For this review, take the finished solid that the model builds, in its own axes (mm). A direction names the side the tool comes from. Coordinates: 2 decimals unless noted, no trailing zeros. Order: outer loops, then holes, each group sorted by start corner. A loop starts at its lowest first (then second) coordinate and runs counter-clockwise, first axis right, second up. Notation, with made-up numbers: (9.5, -9) - (45.5, -9) arc R26 cw to (45.5, 9) - close; hole circle Ø4 at (-10.75, 52). An arc over 180 degrees is marked (long way). One line per item, written item: value. Start each with the question number.
(1) Clearance check with flat-ended pins moving along their axes: pin 1 (9.5 mm diameter, centred on x = 48.26, z = -17.78, fed in from +Y); pin 2 (6 mm diameter, centred on y = 10.5, z = -29, fed in from +X); pin 3 (3 mm diameter, centred on x = 24, y = 5, fed in from -Z); pin 4 (6 mm diameter, centred on y = 10.5, z = -70.5, fed in from +X) (3 decimals). State where each tip first meets the part, or that it passes through.
(2) For faces 4 (the flat face through (0, 9, -149)), 5 (the flat face through (2.9, 8.757, -136.536)), list the 3-axis set-ups (+Z, -Z, +X, -X, +Y, -Y) from which the entire face can be reached by the end or side of a thin tool; tool diameter is ignored.
(3) Consider section D-D on x = 48.26. Write out the cut boundary in (y, z).
(4) Consider section B-B on x = 17.78. Write out the cut boundary in (y, z), then the cut area to 3 significant figures.
(5) Mouldability with a two-part tool opening along Z and no side actions: class faces 1 (the flat face through (38.11, 8.52, -91.42)), 2 (the flat face through (0, 9, -25)), 3 (the cylindrical face through (51.865, 8.757, -21.711)) as released by +Z, released by -Z, zero draft, split by the parting line, or undercut.
(6) To check wall thickness, follow line 1 along X through (y, z) = (4.5, -17.78); line 2 along Z through (x, y) = (4.5, 12); line 3 along Z through (x, y) = (44, 6.25). State the ranges of each line that lie inside material, in increasing order.
(7) Consider section A-A on y = 5.75. Write out the cut boundary in (x, z).
(8) Consider section C-C on z = -17.78. Write out the cut boundary in (x, y), then the cut area to 3 significant figures.
```python
from build123d import *

# Parameters (mm, degrees)
BOSS_EXTRUDE1_DEPTH = 8.636
SKETCH3_R           = 2.667
CUT_EXTRUDE1_DEPTH  = 19.05
FILLET1_R           = 12.7
FILLET2_R           = 2.54
FILLET3_R           = 7.62
CUT_EXTRUDE2_DEPTH  = 84.000499974
SCALE1_SCALE        = 2


with BuildPart() as part:
    # Sketch1 → Boss-Extrude1 (new body)
    with BuildSketch(Plane(origin=(0, 0, 0), x_dir=(1, 0, 0), z_dir=(0, 1, 0))):
        with BuildLine():
            Line((0, 0), (38.1, 0))
            Line((38.1, 0), (6.35, 76.2))
            Line((6.35, 76.2), (0, 76.2))
            Line((0, 76.2), (0, 59.198824612))
            ThreePointArc((0, 59.198824612), (7.62, 38.1), (0, 17.001175388))
            Line((0, 17.001175388), (0, 0))
        make_face()
    extrude(amount=BOSS_EXTRUDE1_DEPTH)

    # Sketch3 → Cut-Extrude1 (cut)
    with BuildSketch(Plane(origin=(0, 8.636, 0), x_dir=(1, 0, 0), z_dir=(0, 1, 0))):
        with Locations(Location((8.89, 8.89, 0), (0, 0, 270))):
            Circle(SKETCH3_R)
        with Locations(Location((24.13, 8.89, 0), (0, 0, 270))):
            Circle(SKETCH3_R)
    extrude(amount=-CUT_EXTRUDE1_DEPTH, mode=Mode.SUBTRACT)

    # Fillet1
    fillet1_edges = [part.edges().sort_by_distance(p)[0] for p in [
        (38.1, 4.318, 0),
    ]]
    fillet(fillet1_edges, radius=FILLET1_R)

    # Fillet2
    fillet2_edges = [part.edges().sort_by_distance(p)[0] for p in [
        (6.35, 4.318, -76.2),
    ]]
    fillet(fillet2_edges, radius=FILLET2_R)

    # Fillet3
    fillet3_edges = [part.edges().sort_by_distance(p)[0] for p in [
        (0, 4.318, 0),
    ]]
    fillet(fillet3_edges, radius=FILLET3_R)

    # Sketch4 → Cut-Extrude2 (cut, through all)
    with BuildSketch(Plane(origin=(0, 8.636, 0), x_dir=(1, 0, 0), z_dir=(0, 1, 0))):
        Polygon((0, 62.500824612), (0, 59.198824612), (2.859615883, 60.849824612), align=None)
        Polygon((0, 65.802824612), (0, 62.500824612), (2.859615883, 64.151824612), align=None)
        Polygon((0, 69.104824612), (0, 65.802824612), (2.859615883, 67.453824612), align=None)
        Polygon((0, 72.406824612), (0, 69.104824612), (2.859615883, 70.755824612), align=None)
    extrude(amount=-CUT_EXTRUDE2_DEPTH, mode=Mode.SUBTRACT)


with BuildPart() as part_1:
    # Scale1: scaled about (0, 0, 0)
    add(part.part.scale(SCALE1_SCALE))


solid = part_1.part
```
Geometry check:
1. pin 1: passes through
1. pin 2: stops at x = 63.49
1. pin 3: stops at z = -128.88
1. pin 4: stops at x = 48.075
2. face 4: +Z, -Z, -X, +Y, -Y
2. face 5: -X, +Y, -Y
3. outline: (0, -67.06) - (17.27, -67.06) - (17.27, -23.11) - (0, -23.11) - close; (0, -12.45) - (17.27, -12.45) - (17.27, -2.12) - (0, -2.12) - close
4. outline: (0, -140.21) - (17.27, -140.21) - (17.27, -23.11) - (0, -23.11) - close; (0, -12.45) - (17.27, -12.45) - (17.27, 0) - (0, 0) - close
4. area: 2,240 mm^2
5. face 1: released by -Z
5. face 2: zero draft
5. face 3: undercut
6. line 1: x = 0 to 12.45, 23.11 to 42.93, 53.59 to 62.33
6. line 2: z = -152.4 to -142.22, -140.81 to -135.61, -134.2 to -129.01, -127.6 to -122.4, -121 to -112.3, -40.1 to -4.43
6. line 3: z = -77.28 to -20.99, -14.57 to -0.69
7. outline: (0, -152.4) - (9.31, -152.4) arc R5.08 ccw to (14, -149.27) - (61.55, -35.17) arc R25.4 ccw to (38.1, 0) - (15.24, 0) arc R15.24 ccw to (0, -15.24) - (0, -34) arc R66.04 cw to (0, -118.4) - (5.72, -121.7) - (0, -125) - (5.72, -128.3) - (0, -131.61) - (5.72, -134.91) - (0, -138.21) - (5.72, -141.51) - (0, -144.81) - close; hole circle Ø10.67 at (17.78, -17.78); hole circle Ø10.67 at (48.26, -17.78)
8. outline: (0, 0) - (12.45, 0) - (12.45, 17.27) - (0, 17.27) - close; (23.11, 0) - (42.93, 0) - (42.93, 17.27) - (23.11, 17.27) - close; (53.59, 0) - (62.33, 0) - (62.33, 17.27) - (53.59, 17.27) - close
8. area: 708 mm^2
